Model file for the job. Use its own axes, mm. A direction names the side the tool comes from. Round coordinates to 2 decimals unless told otherwise and drop trailing zeros. Order: outer loops, then holes, each group sorted by start corner. A loop starts at its lowest first (then second) coordinate and runs counter-clockwise, first axis right, second up. Notation, with made-up numbers: (25, 64.25) - (65, 64.25) arc R19 cw to (65, 98.25) - close; hole circle Ø1 at (86, 42). An arc over 180 degrees is marked (long way). Put each result on its own line as item: value. Start each with the question number.
Item 1: Saw through at C-C on y = -50. State how many separate pieces and enclosed holes the cut face has, plus the area to 3 significant figures.
Item 2: Which spindle directions (+Z, -Z, +X, -X, +Y, -Y) get a long thin tool onto all of the face, cutting with end or side? Do faces 5 (the face through (6, -50, 496)), 6 (the face through (2.958, -48.926, 834.372)). Say none if no direction does.
Item 3: Saw through at A-A on z = 702.5. List the corners of the cut face in (x, y), plus the area to 3 significant figures.
Item 4: Mould opens along Z. For faces 1 (the face through (2.958, -48.926, 774.372)), 2 (the face through (4.513, -46.063, 115.705)), 3 (the face through (2.958, -48.926, 214.372)), 4 (the face through (25, -100, 496)) say: pulls with the +Z half, pulls with the -Z half, needs draft (parallel to the pull), parting line crosses it, or undercut.
Item 5: Probe probe 1 along Y at (x, z) = (13.5, 350); probe 2 along Y at (x, z) = (45.5, 783); probe 3 along X at (y, z) = (-63.5, 152). List the from-to ranges inside material, lowest first.
Item 6: Pin check, flat tips, straight feed: pin 1 Ø15 at (y, z) = (-50, 326.19) entering from -X; pin 2 Ø5 at (y, z) = (-77.5, 489) entering from +X. Stop position of each tip, or through.
Item 7: Saw through at B-B on x = 34.5. List the corners of the cut face in (y, z).
```python
from build123d import *

# Parameters (mm, degrees)
BOSS_EXTRUDE1_DEPTH = 1000
CUT_EXTRUDE4_DEPTH  = 100
SKETCH6_R           = 8.25
CUT_EXTRUDE5_DEPTH  = 100


with BuildPart() as part:
    # Sketch1 → Boss-Extrude1 (new body)
    with BuildSketch(Plane.XY):
        with BuildLine():
            Line((0, 0), (0, -100))
            Line((0, -100), (50, -100))
            Line((50, -100), (50, -98.925311188))
            ThreePointArc((50, -98.925311188), (48.896193111, -95.973045557), (46.126278954, -94.469104878))
            Line((46.126278954, -94.469104878), (13.317028642, -89.858065454))
            ThreePointArc((13.317028642, -89.858065454), (8.084968568, -87.017288616), (6, -81.440786869))
            Line((6, -81.440786869), (6, -18.559213131))
            ThreePointArc((6, -18.559213131), (8.084968568, -12.982711384), (13.317028642, -10.141934546))
            Line((13.317028642, -10.141934546), (46.126278954, -5.530895122))
            ThreePointArc((46.126278954, -5.530895122), (48.896193111, -4.026954443), (50, -1.074688812))
            Line((50, -1.074688812), (50, 0))
            Line((50, 0), (0, 0))
        make_face()
    extrude(amount=BOSS_EXTRUDE1_DEPTH)

    # Sketch5 → Cut-Extrude4 (cut)
    with BuildSketch(Plane(origin=(0, 0, 0), x_dir=(1, 0, 0), z_dir=(0, 1, 0))):
        Polygon((0, -111.192266245), (155.007948876, -266.200215121), (155.007948876, 58.518788552), (-221.01044115, 43.925946333), align=None)
        Polygon((197.398911987, -693.793354258), (279.115957405, -1211.070261728), (0, -1168.351944778), (-115.400263834, -952.431807993), (0, -891.192266245), align=None)
    extrude(amount=-CUT_EXTRUDE4_DEPTH, mode=Mode.SUBTRACT)

    # Sketch6 → Cut-Extrude5 (cut)
    with BuildSketch(Plane.ZY):
        with Locations(Location((146.192266245, -50, 0), (0, 0, 270))):
            Circle(SKETCH6_R)
        with Locations(Location((176.192266245, -50, 0), (0, 0, 270))):
            Circle(SKETCH6_R)
        with Locations(Location((206.192266245, -50, 0), (0, 0, 270))):
            Circle(SKETCH6_R)
        with Locations(Location((236.192266245, -50, 0), (0, 0, 270))):
            Circle(SKETCH6_R)
        with Locations(Location((266.192266245, -50, 0), (0, 0, 270))):
            Circle(SKETCH6_R)
        with Locations(Location((326.192266245, -50, 0), (0, 0, 270))):
            Circle(SKETCH6_R)
        with Locations(Location((676.192266245, -50, 0), (0, 0, 270))):
            Circle(SKETCH6_R)
        with Locations(Location((736.192266245, -50, 0), (0, 0, 270))):
            Circle(SKETCH6_R)
        with Locations(Location((766.192266245, -50, 0), (0, 0, 270))):
            Circle(SKETCH6_R)
        with Locations(Location((796.192266245, -50, 0), (0, 0, 270))):
            Circle(SKETCH6_R)
        with Locations(Location((826.192266245, -50, 0), (0, 0, 270))):
            Circle(SKETCH6_R)
        with Locations(Location((856.192266245, -50, 0), (0, 0, 270))):
            Circle(SKETCH6_R)
    extrude(amount=-CUT_EXTRUDE5_DEPTH, mode=Mode.SUBTRACT)


solid = part.part
```
Results found:
1. separate pieces: 13
1. enclosed holes: 0
1. area: 3,460 mm²
2. face 5: +Z, -Z, +X
2. face 6: +X, -X
3. outline: (0, -100) - (50, -100) - (50, -98.93) arc R4.5 ccw to (46.13, -94.47) - (13.32, -89.86) arc R8.5 cw to (6, -81.44) - (6, -18.56) arc R8.5 cw to (13.32, -10.14) - (46.13, -5.53) arc R4.5 ccw to (50, -1.07) - (50, 0) - (0, 0) - close
3. area: 1,330 mm²
4. face 1: undercut
4. face 2: pulls with the -Z half
4. face 3: undercut
4. face 4: needs draft
5. probe 1: y = -100 to -89.88, -10.12 to 0
5. probe 2: y = -100 to -94.38, -5.62 to 0
5. probe 3: x = 0 to 6
6. pin 1: passes through
6. pin 2: stops at x = 6
7. outline: (-100, 145.69) - (-92.84, 145.69) - (-92.84, 856.69) - (-100, 856.69) - close; (-7.16, 145.69) - (0, 145.69) - (0, 856.69) - (-7.16, 856.69) - close
